Design review of the part shown in the three views and the two pictorial views. Dimensions are in mm from the part's minimum x, y and z. Round coordinates to 2 decimals unless told otherwise and drop trailing zeros. Order: outer loops, then holes, each group sorted by start corner. A loop starts at its lowest first (then second) coordinate and runs counter-clockwise, first axis right, second up. Notation, with made-up numbers: (-8.75, 59) - (47.25, 59) arc R15 ccw to (47.25, 64) - close; hole circle Ø2 at (59.5, -26). An arc over 180 degrees is marked (long way). One line per item, written item: value.
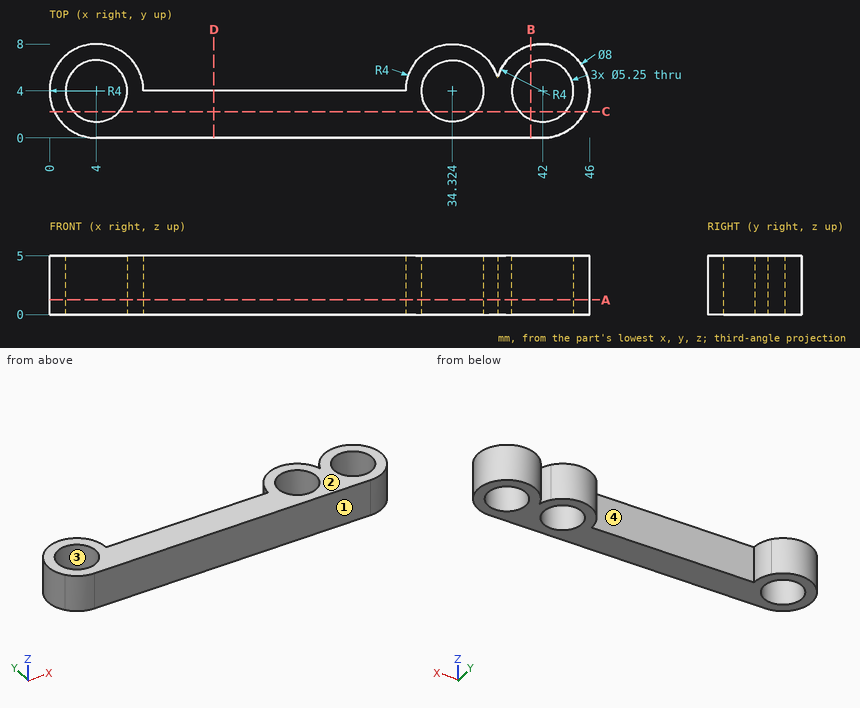
Item 1: Wall thickness on line 1 (Y direction, x = 42, z = 2.05) (3 decimals); line 2 (X direction, y = 5.5, z = 3.55); line 3 (X direction, y = 5, z = 4.25): over which ranges is each line inside the solid? List them lowest first.
Returned:
line 1: 0 to 1.375, 6.625 to 8
line 2: 0.29 to 1.85, 6.15 to 7.71, 30.62 to 32.17, 36.48 to 38.03, 38.29 to 39.85, 44.15 to 45.71
line 3: 0.13 to 1.57, 6.43 to 7.87, 30.45 to 31.9, 36.75 to 39.57, 44.43 to 45.87
Item 2: Take a section at B-B (x = 41). Write out the cut boundary in (y, z).
Returned:
outline: (0, 0) - (1.57, 0) - (1.57, 5) - (0, 5) - close; (6.43, 0) - (7.87, 0) - (7.87, 5) - (6.43, 5) - close
Item 3: Take a section at D-D (x = 14). Write out the cut boundary in (y, z), plus the area to 3 significant figures.
Returned:
outline: (0, 0) - (4, 0) - (4, 5) - (0, 5) - close
area: 20.0 mm^2
Item 4: Take a section at A-A (z = 1.25). Count the separate pieces of the cut face and the enclosed holes in it, plus the area to 3 significant figures.
Returned:
separate pieces: 1
enclosed holes: 3
area: 187 mm^2
Item 5: The part is to be moulded in two halves that separate along Y. For the marked faces 1, 2, 3 and 4, say which applies: +Y half, -Y half, draft (parallel to the pull), parting line (faces both ways), or undercut.
Returned:
face 1: -Y half
face 2: draft
face 3: undercut
face 4: +Y half
Item 6: Take a section at C-C (y = 2.25). Write out the cut boundary in (x, z).
Returned:
outline: (0.4, 0) - (2.04, 0) - (2.04, 5) - (0.4, 5) - close; (5.96, 0) - (32.37, 0) - (32.37, 5) - (5.96, 5) - close; (36.28, 0) - (40.04, 0) - (40.04, 5) - (36.28, 5) - close; (43.96, 0) - (45.6, 0) - (45.6, 5) - (43.96, 5) - close
